```python
from build123d import *

# Parameters (mm, degrees)
SKETCH_1_W          = 10
SKETCH_1_H          = 20
SKETCH_2_R          = 6
EXTRUDE_1_DEPTH     = 224.7
CUT_EXTRUDE_START   = -4.7
CUT_EXTRUDE_1_DEPTH = 4.7
CUT_EXTRUDE_2_DEPTH = 4.7
SKETCH_5_R          = 4.1
EXTRUDE_2_DEPTH     = 1.5
SKETCH_6_R          = 4.1
EXTRUDE_3_DEPTH     = 2.472729678
EXTRUDE_3_DRAFT     = -20
SKETCH_7_R          = 5
EXTRUDE_4_DEPTH     = 15.027270322
DRAFT_1_ANGLE       = 30
DRAFT_2_ANGLE       = 30
CHAMFER_1_SIZE      = 0.767
FILLET_1_R          = 0.6


with BuildPart() as part:
    # 草图1 → 旋转1 (revolve)
    with BuildSketch(Plane(origin=(0, 0, 0), x_dir=(-1, 0, 0), z_dir=(0, 0, -1)), mode=Mode.PRIVATE) as revolve_1_sk:
        with Locations((-223.6, 10)):
            Rectangle(SKETCH_1_W, SKETCH_1_H)
    revolve(revolve_1_sk.sketch.rotate(Axis((228.6, 0, 0), (-1, 0, 0)), 270), axis=Axis((228.6, 0, 0), (-1, 0, 0)))

    # 草图2 → 凸台-拉伸1 (add)
    with BuildSketch(Plane.ZY.offset(-218.6)):
        Circle(SKETCH_2_R)
    extrude(amount=EXTRUDE_1_DEPTH)

    # 草图3 → 切除-拉伸1 (cut)
    with BuildSketch(Plane.ZY.offset(6.1).offset(CUT_EXTRUDE_START)):
        with BuildLine():
            Line((-3.31662479, 5), (3.31662479, 5))
            ThreePointArc((3.31662479, 5), (0, 6), (-3.31662479, 5))
        make_face()
    extrude(amount=CUT_EXTRUDE_1_DEPTH, mode=Mode.SUBTRACT)

    # 草图4 → 切除-拉伸2 (cut)
    with BuildSketch(Plane.ZY.offset(6.1).offset(CUT_EXTRUDE_START)):
        with BuildLine():
            Line((3.31662479, -5), (-3.31662479, -5))
            ThreePointArc((-3.31662479, -5), (0, -6), (3.31662479, -5))
        make_face()
    extrude(amount=CUT_EXTRUDE_2_DEPTH, mode=Mode.SUBTRACT)

    # 草图5 → 凸台-拉伸2 (add)
    with BuildSketch(Plane.ZY.offset(6.1)):
        Circle(SKETCH_5_R)
    extrude(amount=EXTRUDE_2_DEPTH)


with BuildPart() as extrude_3_tool:
    # 草图6 → 凸台-拉伸3 (with draft: the straight prism first)
    with BuildSketch(Plane.ZY.offset(7.6)):
        Circle(SKETCH_6_R)
    extrude(amount=EXTRUDE_3_DEPTH)
    # 凸台-拉伸3: the draft: its side faces are tilted about the plane it starts from
    extrude_3_sides = [extrude_3_tool.faces().sort_by_distance(p)[0] for p in [
        (-8.836364839, 0, -4.1),
    ]]
    draft(extrude_3_sides, Plane.ZY.offset(7.6), EXTRUDE_3_DRAFT)


with BuildPart() as part_1:
    add(part.part)

    # 凸台-拉伸3: add extrude_3_tool
    add(extrude_3_tool.part)

    # 草图7 → 凸台-拉伸4 (add)
    with BuildSketch(Plane.ZY.offset(10.072729678)):
        with Locations(Location((0, 0, 0), (0, 0, 180))):
            Circle(SKETCH_7_R)
    extrude(amount=EXTRUDE_4_DEPTH)

    # 拔模1
    draft_1_faces = [part_1.faces().sort_by_distance(p)[0] for p in [
        (-1.4, -5.403002256, 0),
    ]]
    draft(draft_1_faces, Plane(origin=(-1.4, -5, 3.31662479), x_dir=(0, 0, -1), z_dir=(0, -1, 0)), DRAFT_1_ANGLE)

    # 拔模2
    draft_2_faces = [part_1.faces().sort_by_distance(p)[0] for p in [
        (-1.4, 5.403002256, 0),
    ]]
    draft(draft_2_faces, Plane(origin=(-1.4, 5, -3.31662479), x_dir=(0, 0, 1), z_dir=(0, 1, 0)), DRAFT_2_ANGLE)

    # 倒角1
    chamfer_1_edges = [part_1.edges().sort_by_distance(p)[0] for p in [
        (-25.1, 0, 5),
    ]]
    chamfer(chamfer_1_edges, length=CHAMFER_1_SIZE)

    # 圆角1
    fillet_1_edges = [part_1.edges().sort_by_distance(p)[0] for p in [
        (-6.1, 0, -4.1),
        (-7.6, 0, -4.1),
    ]]
    fillet(fillet_1_edges, radius=FILLET_1_R)


solid = part_1.part
```
Verification items for the finished model (mm, model axes). A direction names the side the tool comes from. Coordinates: 2 decimals unless noted, no trailing zeros. Loops run counter-clockwise (first coordinate to the right, second up) from the corner with the lowest first, then second, coordinate; pieces in that order, holes last. Notation, with made-up numbers: (46.25, -6) -> (97.25, -6) arc R34 ccw to (97.25, 29) -> close; hole circle Ø3 at (21.5, 22). An arc over 180 degrees is marked (long way). Put each result on its own line as item: value.
1. Section check A-A, the plane z = 12. Record the boundary of the cut face in (x, y), then the cut area to 3 significant figures.
Result set:
outline: (218.6, -16) -> (228.6, -16) -> (228.6, 16) -> (218.6, 16) -> close
area: 320 mm^2
2. Gauge pin test, flat ends, axial feed: P1, Ø12, axis at x = 169, y = 4.5, coming from the -Z side; P2, Ø4, axis at y = 9, z = -2.5, coming from the -X side; P3, Ø6, axis at x = 82, y = 10, coming from the -Z side; P4, Ø20, axis at y = -6, z = 5, coming from the -X side. Record the tip position at first contact, or that the pin passes through.
Result set:
P1: stops at z = -6
P2: stops at x = 218.6
P3: passes through
P4: stops at x = -25.1
3. Tool access check on faces 1 (the face through (-7.09, 1.23, 3.91)), 2 (the face through (-4, -5, 0)), 3 (the face through (108, 0, -6)). Record the directions out of +Z, -Z, +X, -X, +Y, -Y that give a thin tool (end or side, any length) a straight path to the whole face; none if there is none.
Result set:
face 1: none
face 2: +Z, -Z, -X, -Y
face 3: -X
4. Section check B-B, the plane x = 36. Record the boundary of the cut face in (y, z).
Result set:
outline: circle Ø12 at (0, 0)
5. Section check C-C, the plane y = 10. Record the boundary of the cut face in (x, z), then the cut area to 3 significant figures.
Result set:
outline: (218.6, -17.32) -> (228.6, -17.32) -> (228.6, 17.32) -> (218.6, 17.32) -> close
area: 346 mm^2
6. Thickness scan on line 1 (X direction, y = -6.5, z = -5.5); line 2 (Z direction, x = 70, y = -1.5); line 3 (Y direction, x = 171, z = -3.5). Record the ranges inside material, lowest first.
Result set:
line 1: x = 218.6 to 228.6
line 2: z = -5.81 to 5.81
line 3: y = -4.87 to 4.87
